Source: CAD feature listing. Evaluate the final solid. Frame: model axes, mm. Face numbers are marked on the shaded views. A direction names the side the tool comes from. Give positions to 0.01 mm unless a question says otherwise; leave off trailing zeros. Write each loop counter-clockwise with the first axis right and the second up, starting at its lowest first coordinate (ties: lowest second). Pieces come first, ordered by that corner, then holes. Notation, with made-up numbers: (-22, 46) - (-4, 46) arc R26 ccw to (-4, 78) - close; hole circle Ø3 at (-1.75, 18.25). An arc over 180 degrees is marked (long way). Answer as a JSON object with one key per item and string values. Group by question number.
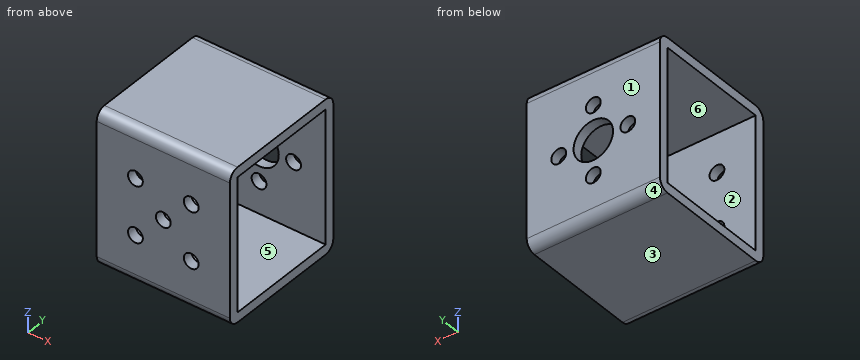
from build123d import *

# Parameters (mm, degrees)
SKETCH1_W           = 27
SKETCH1_H           = 27
BOSS_EXTRUDE1_DEPTH = 29
SKETCH2_W           = 27
SKETCH2_H           = 23
CUT_EXTRUDE1_DEPTH  = 27
CUT_EXTRUDE2_REACH  = 43.86
SKETCH4_R           = 4
SKETCH4_R_2         = 1.5
CUT_EXTRUDE3_REACH  = 43.86
SKETCH5_R           = 1.5
FILLET1_R           = 2
SKETCH6_W           = 27
SKETCH6_H           = 2
BOSS_EXTRUDE2_DEPTH = 27
FILLET2_R           = 2


with BuildPart() as part:
    # Sketch1 → Boss-Extrude1 (new body)
    with BuildSketch(Plane.XY):
        Rectangle(SKETCH1_W, SKETCH1_H)
    extrude(amount=BOSS_EXTRUDE1_DEPTH)

    # Sketch2 → Cut-Extrude1 (cut)
    with BuildSketch(Plane(origin=(13.5, 0, 0), x_dir=(0, 0, -1), z_dir=(1, 0, 0))):
        with Locations((-15.5, 0)):
            Rectangle(SKETCH2_W, SKETCH2_H)
    extrude(amount=-CUT_EXTRUDE1_DEPTH, mode=Mode.SUBTRACT)

    # Sketch4 → Cut-Extrude2 (cut, up to next)
    with BuildSketch(Plane(origin=(0, 13.5, 0), x_dir=(1, 0, 0), z_dir=(0, 1, 0)), mode=Mode.PRIVATE) as cut_extrude2_sk1:
        with Locations(Location((0, -15.5, 0), (0, 0, 270))):
            Circle(SKETCH4_R)
    cut_extrude2_tool1 = extrude(cut_extrude2_sk1.sketch, amount=-CUT_EXTRUDE2_REACH, mode=Mode.PRIVATE) & part.part
    # Sketch4 → Cut-Extrude2 (cut, up to next)
    with BuildSketch(Plane(origin=(0, 13.5, 0), x_dir=(1, 0, 0), z_dir=(0, 1, 0)), mode=Mode.PRIVATE) as cut_extrude2_sk2:
        with Locations(Location((0, -8.5, 0), (0, 0, 270))):
            Circle(SKETCH4_R_2)
    cut_extrude2_tool2 = extrude(cut_extrude2_sk2.sketch, amount=-CUT_EXTRUDE2_REACH, mode=Mode.PRIVATE) & part.part
    # Sketch4 → Cut-Extrude2 (cut, up to next)
    with BuildSketch(Plane(origin=(0, 13.5, 0), x_dir=(1, 0, 0), z_dir=(0, 1, 0)), mode=Mode.PRIVATE) as cut_extrude2_sk3:
        with Locations(Location((7, -15.5, 0), (0, 0, 270))):
            Circle(SKETCH4_R_2)
    cut_extrude2_tool3 = extrude(cut_extrude2_sk3.sketch, amount=-CUT_EXTRUDE2_REACH, mode=Mode.PRIVATE) & part.part
    # Sketch4 → Cut-Extrude2 (cut, up to next)
    with BuildSketch(Plane(origin=(0, 13.5, 0), x_dir=(1, 0, 0), z_dir=(0, 1, 0)), mode=Mode.PRIVATE) as cut_extrude2_sk4:
        with Locations(Location((0, -22.5, 0), (0, 0, 270))):
            Circle(SKETCH4_R_2)
    cut_extrude2_tool4 = extrude(cut_extrude2_sk4.sketch, amount=-CUT_EXTRUDE2_REACH, mode=Mode.PRIVATE) & part.part
    # Sketch4 → Cut-Extrude2 (cut, up to next)
    with BuildSketch(Plane(origin=(0, 13.5, 0), x_dir=(1, 0, 0), z_dir=(0, 1, 0)), mode=Mode.PRIVATE) as cut_extrude2_sk5:
        with Locations(Location((-7, -15.5, 0), (0, 0, 270))):
            Circle(SKETCH4_R_2)
    cut_extrude2_tool5 = extrude(cut_extrude2_sk5.sketch, amount=-CUT_EXTRUDE2_REACH, mode=Mode.PRIVATE) & part.part
    add(cut_extrude2_tool1.solids().sort_by_distance((0, 13.5, 15.5))[0], mode=Mode.SUBTRACT)
    add(cut_extrude2_tool2.solids().sort_by_distance((0, 13.5, 8.5))[0], mode=Mode.SUBTRACT)
    add(cut_extrude2_tool3.solids().sort_by_distance((7, 13.5, 15.5))[0], mode=Mode.SUBTRACT)
    add(cut_extrude2_tool4.solids().sort_by_distance((0, 13.5, 22.5))[0], mode=Mode.SUBTRACT)
    add(cut_extrude2_tool5.solids().sort_by_distance((-7, 13.5, 15.5))[0], mode=Mode.SUBTRACT)

    # Sketch5 → Cut-Extrude3 (cut, up to next)
    with BuildSketch(Plane.XZ.offset(13.5), mode=Mode.PRIVATE) as cut_extrude3_sk1:
        with Locations(Location((0, 15.5, 0), (0, 0, 270))):
            Circle(SKETCH5_R)
    cut_extrude3_tool1 = extrude(cut_extrude3_sk1.sketch, amount=-CUT_EXTRUDE3_REACH, mode=Mode.PRIVATE) & part.part
    # Sketch5 → Cut-Extrude3 (cut, up to next)
    with BuildSketch(Plane.XZ.offset(13.5), mode=Mode.PRIVATE) as cut_extrude3_sk2:
        with Locations(Location((-5.656854249, 21.156854249, 0), (0, 0, 270))):
            Circle(SKETCH5_R)
    cut_extrude3_tool2 = extrude(cut_extrude3_sk2.sketch, amount=-CUT_EXTRUDE3_REACH, mode=Mode.PRIVATE) & part.part
    # Sketch5 → Cut-Extrude3 (cut, up to next)
    with BuildSketch(Plane.XZ.offset(13.5), mode=Mode.PRIVATE) as cut_extrude3_sk3:
        with Locations(Location((5.656854249, 21.156854249, 0), (0, 0, 270))):
            Circle(SKETCH5_R)
    cut_extrude3_tool3 = extrude(cut_extrude3_sk3.sketch, amount=-CUT_EXTRUDE3_REACH, mode=Mode.PRIVATE) & part.part
    # Sketch5 → Cut-Extrude3 (cut, up to next)
    with BuildSketch(Plane.XZ.offset(13.5), mode=Mode.PRIVATE) as cut_extrude3_sk4:
        with Locations(Location((5.656854249, 9.843145751, 0), (0, 0, 270))):
            Circle(SKETCH5_R)
    cut_extrude3_tool4 = extrude(cut_extrude3_sk4.sketch, amount=-CUT_EXTRUDE3_REACH, mode=Mode.PRIVATE) & part.part
    # Sketch5 → Cut-Extrude3 (cut, up to next)
    with BuildSketch(Plane.XZ.offset(13.5), mode=Mode.PRIVATE) as cut_extrude3_sk5:
        with Locations(Location((-5.656854249, 9.843145751, 0), (0, 0, 270))):
            Circle(SKETCH5_R)
    cut_extrude3_tool5 = extrude(cut_extrude3_sk5.sketch, amount=-CUT_EXTRUDE3_REACH, mode=Mode.PRIVATE) & part.part
    add(cut_extrude3_tool1.solids().sort_by_distance((0, -13.5, 15.5))[0], mode=Mode.SUBTRACT)
    add(cut_extrude3_tool2.solids().sort_by_distance((-5.656854, -13.5, 21.156854))[0], mode=Mode.SUBTRACT)
    add(cut_extrude3_tool3.solids().sort_by_distance((5.656854, -13.5, 21.156854))[0], mode=Mode.SUBTRACT)
    add(cut_extrude3_tool4.solids().sort_by_distance((5.656854, -13.5, 9.843146))[0], mode=Mode.SUBTRACT)
    add(cut_extrude3_tool5.solids().sort_by_distance((-5.656854, -13.5, 9.843146))[0], mode=Mode.SUBTRACT)

    # Fillet1
    fillet1_edges = [part.edges().sort_by_distance(p)[0] for p in [
        (0, -13.5, 0),
        (0, 13.5, 0),
    ]]
    fillet(fillet1_edges, radius=FILLET1_R)

    # Sketch6 → Boss-Extrude2 (add)
    with BuildSketch(Plane.XZ.offset(13.5)):
        with Locations((0, 30)):
            Rectangle(SKETCH6_W, SKETCH6_H)
    extrude(amount=-BOSS_EXTRUDE2_DEPTH)

    # Fillet2
    fillet2_edges = [part.edges().sort_by_distance(p)[0] for p in [
        (0, -13.5, 31),
        (0, 13.5, 31),
    ]]
    fillet(fillet2_edges, radius=FILLET2_R)


solid = part.part
Q1. Section B-B on x = 0. Return the cut outline in (y, z), then the cut area to 3 significant figures.
Q2. Section C-C on y = 4.75. Return the cut outline in (x, z), then the cut area to 3 significant figures.
Q3. Ray query, probe 1 along X at (y, z) = (12.9, 15.5); probe 2 along Z at (x, y) = (5.25, -4.25); probe 3 along X at (y, z) = (12, 8.5). Return the intervals inside material, ascending. Write a range as [from, to].
Q4. Section D-D on z = 9.5. Return the cut outline in (x, y), then the cut area to 3 significant figures.
Q5. Section A-A on z = 27.5. Return the cut outline in (x, y), then the cut area to 3 significant figures.
Q6. First-contact query: pin 1 Ø7 at (x, z) = (0, 15.5) entering from +Y; pin 2 Ø2.5 at (x, z) = (-5.66, 9.84) entering from -Y. Flat tips, straight axial feed; report the tip coordinate or a pass-through.
Q7. Reachability of the marked faces 1 and 2 from +Z, -Z, +X, -X, +Y, -Y: full face, straight path, thin tool, end or side. Return the list, or none.
Q8. Draft query along Y for the marked faces 3, 4, 5 and 6. Return one class per face: released by +Y, released by -Y, zero draft, split by the parting line, or undercut.
Taken from the geometry:
{
 "1": {"outline": "(-13.5, 2) arc R2 ccw to (-11.5, 0) - (11.5, 0) arc R2 ccw to (13.5, 2) - (13.5, 7) - (11.5, 7) - (11.5, 2) - (-11.5, 2) - (-11.5, 14) - (-13.5, 14) - close; (-13.5, 17) - (-11.5, 17) - (-11.5, 29) - (11.5, 29) - (11.5, 24) - (13.5, 24) - (13.5, 29) arc R2 ccw to (11.5, 31) - (-11.5, 31) arc R2 ccw to (-13.5, 29) - close; (11.5, 10) - (13.5, 10) - (13.5, 11.5) - (11.5, 11.5) - close; (11.5, 19.5) - (13.5, 19.5) - (13.5, 21) - (11.5, 21) - close", "area": "179 mm²"},
 "2": {"outline": "(-13.5, 0) - (13.5, 0) - (13.5, 2) - (-13.5, 2) - close; (-13.5, 29) - (13.5, 29) - (13.5, 31) - (-13.5, 31) - close", "area": "108 mm²"},
 "3": {"probe 1": "x = [-13.5, -8.5], [-5.5, -4], [4, 5.5], [8.5, 13.5]", "probe 2": "z = [0, 2], [29, 31]", "probe 3": "x = [-13.5, -1.5], [1.5, 13.5]"},
 "4": {"outline": "(-13.5, -13.5) - (-7.12, -13.5) - (-7.12, -11.5) - (-13.5, -11.5) - close; (-13.5, 11.5) - (-1.12, 11.5) - (-1.12, 13.5) - (-13.5, 13.5) - close; (-4.2, -13.5) - (4.2, -13.5) - (4.2, -11.5) - (-4.2, -11.5) - close; (1.12, 11.5) - (13.5, 11.5) - (13.5, 13.5) - (1.12, 13.5) - close; (7.12, -13.5) - (13.5, -13.5) - (13.5, -11.5) - (7.12, -11.5) - close", "area": "91.8 mm²"},
 "5": {"outline": "(-13.5, -13.5) - (13.5, -13.5) - (13.5, -11.5) - (-13.5, -11.5) - close; (-13.5, 11.5) - (13.5, 11.5) - (13.5, 13.5) - (-13.5, 13.5) - close", "area": "108 mm²"},
 "6": {"pin 1": "stops at y = -11.5", "pin 2": "stops at y = 11.5"},
 "7": {"face 1": "+Z, -Z, +X, -X, +Y", "face 2": "+X, -X"},
 "8": {"face 3": "zero draft", "face 4": "released by +Y", "face 5": "undercut", "face 6": "undercut"}
}
